CAD build for the part. Positions are in the model's coordinates, mm. A direction names the side the tool comes from. Give positions to 0.01 mm unless a question says otherwise; leave off trailing zeros. Order: outer loops, then holes, each group sorted by start corner. A loop starts at its lowest first (then second) coordinate and runs counter-clockwise, first axis right, second up.
from build123d import *

# Parameters (mm, degrees)
BOSS_EXTRUDE1_DEPTH = 20
BOSS_EXTRUDE2_DEPTH = 1431
BOSS_EXTRUDE3_DEPTH = 25
BOSS_EXTRUDE4_START = -30
BOSS_EXTRUDE4_DEPTH = 15
BOSS_EXTRUDE7_START = -30
BOSS_EXTRUDE7_DEPTH = 15


with BuildPart() as part:
    # Sketch1 → Boss-Extrude1 (new body)
    with BuildSketch(Plane(origin=(0, 0, 0), x_dir=(1, 0, 0), z_dir=(0, 1, 0))):
        Polygon((0, 310), (10, 320), (410, 320), (420, 310), (420, 10), (410, 0), (10, 0), (0, 10), align=None)
    extrude(amount=BOSS_EXTRUDE1_DEPTH)

    # Sketch2 → Boss-Extrude2 (add)
    with BuildSketch(Plane(origin=(0, 20, 0), x_dir=(1, 0, 0), z_dir=(0, 1, 0))):
        with BuildLine():
            Line((79.070897456, 260), (340.929102544, 260))
            ThreePointArc((340.929102544, 260), (354.414263459, 254.414263459), (360, 240.929102544))
            Line((360, 240.929102544), (360, 79.070897456))
            ThreePointArc((360, 79.070897456), (354.414263459, 65.585736541), (340.929102544, 60))
            Line((340.929102544, 60), (79.070897456, 60))
            ThreePointArc((79.070897456, 60), (65.585736541, 65.585736541), (60, 79.070897456))
            Line((60, 79.070897456), (60, 240.929102544))
            ThreePointArc((60, 240.929102544), (65.585736541, 254.414263459), (79.070897456, 260))
        make_face()
        with BuildLine():
            Line((79.070897456, 252), (340.929102544, 252))
            ThreePointArc((340.929102544, 252), (348.757409209, 248.757409209), (352, 240.929102544))
            Line((352, 240.929102544), (352, 79.070897456))
            ThreePointArc((352, 79.070897456), (348.757409209, 71.242590791), (340.929102544, 68))
            Line((340.929102544, 68), (79.070897456, 68))
            ThreePointArc((79.070897456, 68), (71.242590791, 71.242590791), (68, 79.070897456))
            Line((68, 79.070897456), (68, 240.929102544))
            ThreePointArc((68, 240.929102544), (71.242590791, 248.757409209), (79.070897456, 252))
        make_face(mode=Mode.SUBTRACT)
    extrude(amount=BOSS_EXTRUDE2_DEPTH)

    # Sketch3 → Boss-Extrude3 (add)
    with BuildSketch(Plane(origin=(0, 1451, 0), x_dir=(1, 0, 0), z_dir=(0, 1, 0))):
        Polygon((-10, 310), (430, 310), (440, 300), (440, 20), (430, 10), (-10, 10), (-20, 20), (-20, 300), align=None)
    extrude(amount=BOSS_EXTRUDE3_DEPTH)

    # Sketch4 → Boss-Extrude4 (add)
    with BuildSketch(Plane(origin=(0, 0, -260), x_dir=(-1, 0, 0), z_dir=(0, 0, -1)).offset(BOSS_EXTRUDE4_START)):
        Polygon((-30, 320), (-10, 50), (-10, 20), (-410, 20), (-410, 50), (-390, 320), align=None)
    boss_extrude4 = extrude(amount=-BOSS_EXTRUDE4_DEPTH)

    # Mirror1: Boss-Extrude4 across plane
    add(boss_extrude4.mirror(Plane.XY.offset(-160)))

    # Sketch5 → Boss-Extrude7 (add)
    with BuildSketch(Plane.XY.offset(-60).offset(BOSS_EXTRUDE7_START)):
        Polygon((60, 1441), (50, 1451), (-10, 1451), (-10, 1421), (30, 1101), (60, 1101), align=None)
    boss_extrude7 = extrude(amount=-BOSS_EXTRUDE7_DEPTH)

    # Mirror5: Boss-Extrude7 across plane
    add(boss_extrude7.mirror(Plane.XY.offset(-160)))


solid = part.part
1. Pin check, flat tips, straight feed: P1, Ø15, axis at x = 33, y = 122.5, coming from the +Z side; P2, Ø10, axis at x = 203, y = 568.5, coming from the +Z side; P3, Ø3, axis at x = 359, y = 495, coming from the +Z side. Stop position of each tip, or through.
2. Mould opens along Y. For faces 1 (the flat face through (213, 1476, -162)), 2 (the flat face through (440, 1463, -162)), 3 (the flat face through (212, 1451, -161)) say: released by +Y, released by -Y, zero draft, split by the parting line, or undercut.
3. Saw through at D-D on y = 1368.5. Give the cut face in (x, z), plus the area to 3 significant figures.
4. Saw through at C-C on x = 271. Give the cut face in (y, z).
5. Saw through at A-A on z = -169. Give the cut face in (x, y), plus the area to 3 significant figures.
6. Wall check: line 1 (Z direction, x = 270, y = 256); line 2 (Y direction, x = 44, z = -67); line 3 (Z direction, x = 216.5, y = 881). Give the ranges that are in metal, low to high.
7. Saw through at B-B on y = 863.5. Give the cut face in (x, z), plus the area to 3 significant figures.
8. 3-axis set-ups, long thin cutter, end or side, ignore diameter. For faces 4 (the flat face through (32, 1317, -105)), 5 (the flat face through (379, 172, -230)), 6 (the flat face through (212, 725, -60)), 7 (the flat face through (9.72, 1263.24, -97.4)), 8 (the flat face through (40, 172, -230)): which of +Z, -Z, +X, -X, +Y, -Y reach the whole face in a straight line?
Reported:
1. P1: stops at z = -90
1. P2: stops at z = -60
1. P3: stops at z = -69.63
2. face 1: released by +Y
2. face 2: zero draft
2. face 3: undercut
3. outline: (-3.44, -230) - (60, -230) - (60, -240.93) arc R19.07 ccw to (79.07, -260) - (340.93, -260) arc R19.07 ccw to (360, -240.93) - (360, -79.07) arc R19.07 ccw to (340.93, -60) - (79.07, -60) arc R19.07 ccw to (60, -79.07) - (60, -90) - (-3.44, -90) - (-3.44, -105) - (60, -105) - (60, -215) - (-3.44, -215) - close; hole (68, -240.93) arc R11.07 ccw to (79.07, -252) - (340.93, -252) arc R11.07 ccw to (352, -240.93) - (352, -79.07) arc R11.07 ccw to (340.93, -68) - (79.07, -68) arc R11.07 ccw to (68, -79.07) - close
3. area: 9,440 mm2
4. outline: (0, -320) - (20, -320) - (20, -260) - (1451, -260) - (1451, -310) - (1476, -310) - (1476, -10) - (1451, -10) - (1451, -60) - (20, -60) - (20, 0) - (0, 0) - close; hole (20, -252) - (1451, -252) - (1451, -68) - (20, -68) - (20, -90) - (320, -90) - (320, -105) - (20, -105) - (20, -215) - (320, -215) - (320, -230) - (20, -230) - close
5. outline: (-20, 1451) - (60, 1451) - (60, 20) - (0, 20) - (0, 0) - (420, 0) - (420, 20) - (360, 20) - (360, 1451) - (440, 1451) - (440, 1476) - (-20, 1476) - close; hole (68, 20) - (352, 20) - (352, 1451) - (68, 1451) - close
5. area: 42,800 mm2
6. line 1: z = -260 to -252, -230 to -215, -105 to -90, -68 to -60
6. line 2: y = 0 to 20, 1451 to 1476
6. line 3: z = -260 to -252, -68 to -60
7. outline: (60, -240.93) arc R19.07 ccw to (79.07, -260) - (340.93, -260) arc R19.07 ccw to (360, -240.93) - (360, -79.07) arc R19.07 ccw to (340.93, -60) - (79.07, -60) arc R19.07 ccw to (60, -79.07) - close; hole (68, -240.93) arc R11.07 ccw to (79.07, -252) - (340.93, -252) arc R11.07 ccw to (352, -240.93) - (352, -79.07) arc R11.07 ccw to (340.93, -68) - (79.07, -68) arc R11.07 ccw to (68, -79.07) - close
7. area: 7,540 mm2
8. face 4: -X
8. face 5: -Z, +X
8. face 6: +Z, +X, -X
8. face 7: +Z, -Z, -X
8. face 8: -Z, -X
